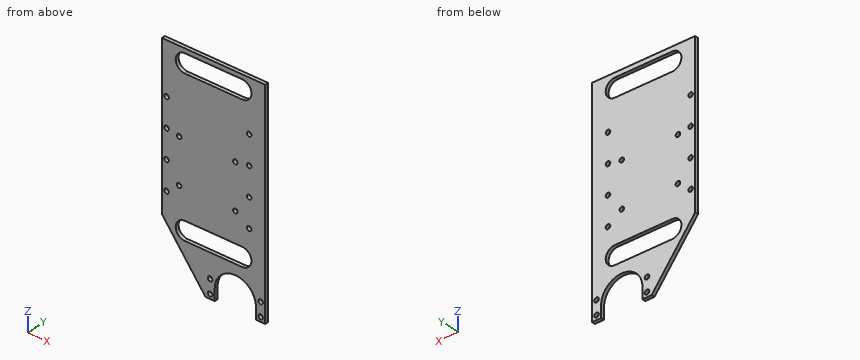
```python
from build123d import *

# Parameters (mm, degrees)
BOSS_EXTRUDE1_DEPTH = 3
SKETCH2_R           = 2
CUT_EXTRUDE1_DEPTH  = 3


with BuildPart() as part:
    # Sketch1 → Boss-Extrude1 (new body)
    with BuildSketch(Plane(origin=(0, 0, 0), x_dir=(1, 0, 0), z_dir=(0, 1, 0))):
        Polygon((-12, -7.26193593), (40, -7.26193593), (40, -197.26193593), (-50, -197.26193593), (-50, -57.26193593), align=None)
    extrude(amount=BOSS_EXTRUDE1_DEPTH)

    # Sketch2 → Cut-Extrude1 (cut)
    with BuildSketch(Plane(origin=(0, 3, 0), x_dir=(1, 0, 0), z_dir=(0, 1, 0))):
        with BuildLine():
            Line((-30, -193.26193593), (20, -193.26193593))
            ThreePointArc((20, -193.26193593), (28, -185.26193593), (20, -177.26193593))
            Line((20, -177.26193593), (-30, -177.26193593))
            ThreePointArc((-30, -177.26193593), (-38, -185.26193593), (-30, -193.26193593))
        make_face()
        with BuildLine():
            Line((-30, -60.26193593), (20, -60.26193593))
            ThreePointArc((20, -60.26193593), (28, -52.26193593), (20, -44.26193593))
            Line((20, -44.26193593), (-30, -44.26193593))
            ThreePointArc((-30, -44.26193593), (-38, -52.26193593), (-30, -60.26193593))
        make_face()
        with BuildLine():
            ThreePointArc((-4, -17.26193593), (14, -35.26193593), (32, -17.26193593))
            Line((32, -17.26193593), (32, -7.26193593))
            Line((32, -7.26193593), (-4, -7.26193593))
            Line((-4, -7.26193593), (-4, -17.26193593))
        make_face()
        with Locations(Location((-46, -152.26193593, 0), (0, 0, 270))):
            Circle(SKETCH2_R)
        with Locations(Location((-46, -77.26193593, 0), (0, 0, 270))):
            Circle(SKETCH2_R)
        with Locations(Location((-46, -127.26193593, 0), (0, 0, 270))):
            Circle(SKETCH2_R)
        with Locations(Location((-46, -102.26193593, 0), (0, 0, 270))):
            Circle(SKETCH2_R)
        with Locations(Location((-8, -11.26193593, 0), (0, 0, 270))):
            Circle(SKETCH2_R)
        with Locations(Location((-8, -23.26193593, 0), (0, 0, 270))):
            Circle(SKETCH2_R)
        with Locations(Location((26, -152.26193593, 0), (0, 0, 270))):
            Circle(SKETCH2_R)
        with Locations(Location((26, -102.26193593, 0), (0, 0, 270))):
            Circle(SKETCH2_R)
        with Locations(Location((26, -127.26193593, 0), (0, 0, 270))):
            Circle(SKETCH2_R)
        with Locations(Location((26, -77.26193593, 0), (0, 0, 270))):
            Circle(SKETCH2_R)
        with Locations(Location((36, -23.26193593, 0), (0, 0, 270))):
            Circle(SKETCH2_R)
        with Locations(Location((36, -11.26193593, 0), (0, 0, 270))):
            Circle(SKETCH2_R)
        with Locations(Location((-35, -86.26193593, 0), (0, 0, 270))):
            Circle(SKETCH2_R)
        with Locations(Location((-35, -125.26193593, 0), (0, 0, 270))):
            Circle(SKETCH2_R)
        with Locations(Location((14, -86.26193593, 0), (0, 0, 270))):
            Circle(SKETCH2_R)
        with Locations(Location((14, -125.26193593, 0), (0, 0, 270))):
            Circle(SKETCH2_R)
    extrude(amount=-CUT_EXTRUDE1_DEPTH, mode=Mode.SUBTRACT)


solid = part.part
```
For this review, take the finished solid that the model builds, in its own axes (mm). Coordinates: 2 decimals unless noted, no trailing zeros. Write each loop counter-clockwise with the first axis right and the second up, starting at its lowest first coordinate (ties: lowest second). Pieces come first, ordered by that corner, then holes. Notation, with made-up numbers: (46, 74.25) - (66, 74.25) arc R17 cw to (66, 104.25) - close; hole circle Ø9 at (-14, -30.75). An arc over 180 degrees is marked (long way). Put each result on its own line as item: value.
1. Add section A-A, the plane x = -8. Give the boundary of the cut face in (y, z), then the cut area to 3 significant figures.
Values found:
outline: (0, 7.26) - (3, 7.26) - (3, 9.26) - (0, 9.26) - close; (0, 13.26) - (3, 13.26) - (3, 21.26) - (0, 21.26) - close; (0, 25.26) - (3, 25.26) - (3, 44.26) - (0, 44.26) - close; (0, 60.26) - (3, 60.26) - (3, 177.26) - (0, 177.26) - close; (0, 193.26) - (3, 193.26) - (3, 197.26) - (0, 197.26) - close
area: 450 mm²
2. Add section B-B, the plane y = 2.25. Count the separate pieces of the cut face and the enclosed holes in it, then the cut area to 3 significant figures.
Values found:
separate pieces: 1
enclosed holes: 18
area: 13,100 mm²
3. Add section C-C, the plane x = 26. Give the boundary of the cut face in (y, z).
Values found:
outline: (0, 30.68) - (3, 30.68) - (3, 46.97) - (0, 46.97) - close; (0, 57.55) - (3, 57.55) - (3, 75.26) - (0, 75.26) - close; (0, 79.26) - (3, 79.26) - (3, 100.26) - (0, 100.26) - close; (0, 104.26) - (3, 104.26) - (3, 125.26) - (0, 125.26) - close; (0, 129.26) - (3, 129.26) - (3, 150.26) - (0, 150.26) - close; (0, 154.26) - (3, 154.26) - (3, 179.97) - (0, 179.97) - close; (0, 190.55) - (3, 190.55) - (3, 197.26) - (0, 197.26) - close
4. Wall thickness on probe 1 along Z at (x, y) = (-9, 1.75); probe 2 along Z at (x, y) = (-11, 1.65); probe 3 along X at (y, z) = (2.05, 152): over which ranges is each line inside the solid? List them lowest first.
Values found:
probe 1: 7.26 to 9.53, 12.99 to 21.53, 24.99 to 44.26, 60.26 to 177.26, 193.26 to 197.26
probe 2: 7.26 to 44.26, 60.26 to 177.26, 193.26 to 197.26
probe 3: -50 to -47.98, -44.02 to 24.02, 27.98 to 40
5. Add section D-D, the plane x = 14. Give the boundary of the cut face in (y, z), then the cut area to 3 significant figures.
Values found:
outline: (0, 35.26) - (3, 35.26) - (3, 44.26) - (0, 44.26) - close; (0, 60.26) - (3, 60.26) - (3, 84.26) - (0, 84.26) - close; (0, 88.26) - (3, 88.26) - (3, 123.26) - (0, 123.26) - close; (0, 127.26) - (3, 127.26) - (3, 177.26) - (0, 177.26) - close; (0, 193.26) - (3, 193.26) - (3, 197.26) - (0, 197.26) - close
area: 366 mm²
